from build123d import *

# Parameters (mm, degrees)
CHAMFER1_SIZE = 0.5


with BuildPart() as part:
    # Sketch1 → Revolve1 (revolve)
    with BuildSketch(Plane.XY, mode=Mode.PRIVATE) as revolve1_sk:
        Polygon((0, 0), (0, 3), (10, 3), (10, 5.25), (11, 5.25), (11, 11), (68.6, 11), (68.6, 4.26180602), (69.6, 4.26180602), (69.6, 2.01180602), (79.6, 2.01180602), (79.6, 0), align=None)
    revolve(revolve1_sk.sketch.rotate(Axis((0, 0, 0), (1, 0, 0)), 90), axis=Axis((0, 0, 0), (1, 0, 0)))

    # Chamfer1
    chamfer1_edges = [part.edges().sort_by_distance(p)[0] for p in [
        (69.6, 0, -4.26180602),
        (68.6, 0, -11),
        (11, 0, -11),
        (10, 0, -5.25),
        (0, 0, -3),
        (79.6, 0, -2.01180602),
    ]]
    chamfer(chamfer1_edges, length=CHAMFER1_SIZE)


solid = part.part
Geometry check sheet. Reference: the model listing, model coordinates, mm. A direction names the side the tool comes from. Give positions to 0.01 mm unless a question says otherwise; leave off trailing zeros. Write each loop counter-clockwise with the first axis right and the second up, starting at its lowest first coordinate (ties: lowest second). Pieces come first, ordered by that corner, then holes.
1) Set-up check for faces 1 (the face through (69.6, 2, 2)), 2 (the face through (40.2, 10.74, -2.38)), 3 (the face through (5.32, -0.9, 2.86)): record each of +Z, -Z, +X, -X, +Y, -Y from which the full face is reachable in a straight line by a thin tool's end or side.
Values follow:
face 1: +X
face 2: +X, -X
face 3: -X
2) Thickness scan on line 1 (Z direction, x = 62, y = 0.5); line 2 (X direction, y = 7.75, z = 7); line 3 (Z direction, x = 22.5, y = -9). Record the ranges inside material, lowest first.
Values follow:
line 1: z = -10.99 to 10.99
line 2: x = 11 to 68.6
line 3: z = -6.32 to 6.32
3) Cross-section at C-C (x = 31). Record the boundary of the cut face in (y, z).
Values follow:
outline: circle Ø22 at (0, 0)
4) Go/stop test with flat-tipped pins: pin 1 Ø1.5 at (x, z) = (17, 3) entering from -Y; pin 2 Ø8 at (x, y) = (36.5, 5.5) entering from +Z; pin 3 Ø4 at (x, y) = (24, -5.5) entering from -Z. Record where each tip stops, or that it passes through.
Values follow:
pin 1: stops at y = -10.77
pin 2: stops at z = 10.9
pin 3: stops at z = -10.43
